```python
from build123d import *

# Parameters (mm, degrees)
EXTRUDE_1_DEPTH     = 50
CUT_EXTRUDE_1_DEPTH = 10


with BuildPart() as part:
    # 草图1 → 拉伸-薄壁1 (new body)
    with BuildSketch(Plane.XY):
        Polygon((0, 0), (0, 60), (120, 60), (120, 55), (5, 55), (5, 0), align=None)
    extrude(amount=EXTRUDE_1_DEPTH)

    # 草图2 → 切除-拉伸1 (cut)
    with BuildSketch(Plane.ZY):
        with BuildLine():
            Line((8, 24.25), (42, 24.25))
            ThreePointArc((42, 24.25), (46.25, 20), (42, 15.75))
            Line((42, 15.75), (8, 15.75))
            ThreePointArc((8, 15.75), (3.75, 20), (8, 24.25))
        make_face()
    extrude(amount=-CUT_EXTRUDE_1_DEPTH, mode=Mode.SUBTRACT)


solid = part.part
```
Part model, mm, in its own coordinate system. A direction names the side the tool comes from. Round coordinates to 2 decimals unless told otherwise and drop trailing zeros. Loops run counter-clockwise (first coordinate to the right, second up) from the corner with the lowest first, then second, coordinate; pieces in that order, holes last.
Item 1: Cut at B-B, the plane z = 29. Give the cut face in (x, y), then the cut area to 4 significant figures.
Item 2: Cut at D-D, the plane x = 110. Give the cut face in (y, z), then the cut area to 3 significant figures.
Item 3: Cut at A-A, the plane y = 20. Give the cut face in (x, z).
Item 4: 3-axis set-ups, long thin cutter, end or side, ignore diameter. For faces 4 (the face through (5, 28, 25)), 5 (the face through (3, 0, 25)), 6 (the face through (2.46, 20.09, 46.25)): which of +Z, -Z, +X, -X, +Y, -Y reach the whole face in a straight line?
Item 5: Drill centre lines: line 1 (X direction, y = 41, z = 40.5); line 2 (Y direction, x = 59.5, z = 35). Where is each one in solid material? Low to high.
Item 6: Drop flat-ended pins along their axis: P1, Ø10, axis at x = 14.5, z = 5, coming from the -Y side; P2, Ø1.5, axis at x = 1.5, z = 18.5, coming from the -Y side; P3, Ø6, axis at y = 46, z = 31, coming from the +X side. Give the stop position or say it passes through.
Item 7: Mould opens along Y. For faces 1 (the face through (2.46, 19.91, 3.75)), 2 (the face through (43, 57, 0)), 3 (the face through (59, 60, 25)) say: +Y half, -Y half, draft (parallel to the pull), parting line (faces both ways), or undercut.
Item 8: Cut at C-C, the plane y = 32.5. Give the cut face in (x, z).
A:
1. outline: (0, 0) - (5, 0) - (5, 15.75) - (0, 15.75) - close; (0, 24.25) - (5, 24.25) - (5, 55) - (120, 55) - (120, 60) - (0, 60) - close
1. area: 832.5 mm2
2. outline: (55, 0) - (60, 0) - (60, 50) - (55, 50) - close
2. area: 250 mm2
3. outline: (0, 0) - (5, 0) - (5, 3.75) - (0, 3.75) - close; (0, 46.25) - (5, 46.25) - (5, 50) - (0, 50) - close
4. face 4: +Z, -Z, +X, -Y
4. face 5: +Z, -Z, +X, -X, -Y
4. face 6: +X, -X
5. line 1: x = 0 to 5
5. line 2: y = 55 to 60
6. P1: stops at y = 55
6. P2: stops at y = 0
6. P3: stops at x = 5
7. face 1: undercut
7. face 2: draft
7. face 3: +Y half
8. outline: (0, 0) - (5, 0) - (5, 50) - (0, 50) - close
